Source: CAD feature listing. Evaluate the final solid. Frame: model axes, mm. A direction names the side the tool comes from. Give positions to 0.01 mm unless a question says otherwise; leave off trailing zeros. Loops run counter-clockwise (first coordinate to the right, second up) from the corner with the lowest first, then second, coordinate; pieces in that order, holes last.
from build123d import *

# Parameters (mm, degrees)
SKETCH_1_W          = 120
SKETCH_1_H          = 15
EXTRUDE_1_DEPTH     = 8
CUT_EXTRUDE_1_DEPTH = 0.3
SKETCH_6_W          = 50
SKETCH_6_H          = 14
EXTRUDE_2_DEPTH     = 15


with BuildPart() as part:
    # 草图1 → 凸台-拉伸1 (new body)
    with BuildSketch(Plane.XY):
        Rectangle(SKETCH_1_W, SKETCH_1_H)
    extrude(amount=EXTRUDE_1_DEPTH)

    # 草图2 → 切除-拉伸1 (cut)
    with BuildSketch(Plane.XY.offset(8)):
        Polygon((50.687670047, 7.5), (52, -7.5), (8.835746986, -7.5), (7.523417033, 7.5), align=None)
    extrude(amount=-CUT_EXTRUDE_1_DEPTH, mode=Mode.SUBTRACT)

    # 草图6 → 凸台-拉伸2 (add)
    with BuildSketch(Plane.XZ.offset(7.5)):
        with Locations((-35, 15)):
            Rectangle(SKETCH_6_W, SKETCH_6_H)
    extrude(amount=-EXTRUDE_2_DEPTH)


solid = part.part
1) Contact query for flat-ended pins moving along their axis: P1, Ø7.5, axis at x = 1.5, y = 1, coming from the +Z side; P2, Ø4, axis at y = 0.5, z = 8.5, coming from the +X side; P3, Ø1.5, axis at y = 1, z = 15, coming from the +X side. Output: stop coordinate, or through.
Checks:
P1: stops at z = 8
P2: stops at x = 60
P3: stops at x = -10
2) Cut plane A-A (y = 0). Return loops of the section in (x, z), and give its area (3 significant figures).
Checks:
outline: (-60, 0) - (60, 0) - (60, 8) - (51.34, 8) - (51.34, 7.7) - (8.18, 7.7) - (8.18, 8) - (-10, 8) - (-10, 22) - (-60, 22) - close
area: 1,650 mm2
3) Cut plane C-C (z = 10). Return loops of the section in (x, y), and give its area (3 significant figures).
Checks:
outline: (-60, -7.5) - (-10, -7.5) - (-10, 7.5) - (-60, 7.5) - close
area: 750 mm2
4) Ray query, probe 1 along X at (y, z) = (-0.75, 11.75); probe 2 along Z at (x, y) = (7.5, -5.5); probe 3 along Z at (x, y) = (38.5, 4.75). Return the intervals inside material, ascending.
Checks:
probe 1: x = -60 to -10
probe 2: z = 0 to 8
probe 3: z = 0 to 7.7
5) Cut plane B-B (x = 43). Return loops of the section in (y, z).
Checks:
outline: (-7.5, 0) - (7.5, 0) - (7.5, 7.7) - (-7.5, 7.7) - close
6) Reachability of faces 1 (the flat face through (60, 0, 4)), 2 (the flat face through (55, 0, 8)) from +Z, -Z, +X, -X, +Y, -Y: full face, straight path, thin tool, end or side. Return the list, or none.
Checks:
face 1: +Z, -Z, +X, +Y, -Y
face 2: +Z, +X, +Y, -Y
